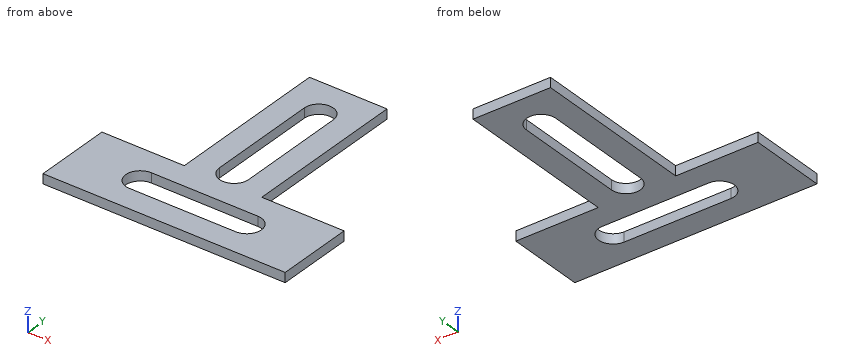
from build123d import *

# Parameters (mm, degrees)
EXTRUDE_2_DEPTH = 2


with BuildPart() as part:
    # 草图1 → 凸台-拉伸2 (new body)
    with BuildSketch(Plane.XY):
        Polygon((25, -8), (-25, -8), (-25, 8), (-8, 8), (-8, 42), (8, 42), (8, 8), (25, 8), align=None)
        with BuildLine():
            Line((-3, 11), (-3, 34))
            ThreePointArc((-3, 34), (0, 37), (3, 34))
            Line((3, 34), (3, 11))
            ThreePointArc((3, 11), (0, 8), (-3, 11))
        make_face(mode=Mode.SUBTRACT)
        with BuildLine():
            Line((-11, 3), (11, 3))
            ThreePointArc((11, 3), (14, 0), (11, -3))
            Line((11, -3), (-11, -3))
            ThreePointArc((-11, -3), (-14, 0), (-11, 3))
        make_face(mode=Mode.SUBTRACT)
    extrude(amount=EXTRUDE_2_DEPTH)


solid = part.part
Can you work these out from the model? Positions are in its coordinate system, mm. Round coordinates to 2 decimals unless told otherwise and drop trailing zeros. Loops run counter-clockwise (first coordinate to the right, second up) from the corner with the lowest first, then second, coordinate; pieces in that order, holes last. Notation, with made-up numbers: (61.5, 81) - (72.5, 81) arc R9 cw to (72.5, 88) - close; hole circle Ø5 at (12.25, 4). An arc over 180 degrees is marked (long way). Write item = value, one per line. Start each with the question number.
(1) If we section it at A-A (y = 30): Please give me the cut outline in (x, z).
(2) If we section it at B-B (z = 0.9): Please give me the cut outline in (x, y), and give its area (3 significant figures).
(3) If we section it at C-C (x = 1.5): Please give me the cut outline in (y, z), and give its area (3 significant figures).
(4) If we section it at D-D (x = 17): Please give me the cut outline in (y, z).
(5) If I drill on probe 1 along X at (y, z) = (34, 1.35); probe 2 along Y at (x, z) = (7, 0.3); probe 3 along Y at (x, z) = (17.5, 1.6), over which ranges is the centre line in solid material (lowest first)? Write a range as [from, to].
(6) For P1, Ø0.6, axis at y = 32, z = 1.5, coming from the +X side; P2, Ø0.6, axis at y = 28, z = 1, coming from the -X side, each with a flat end and sliding along its axis, tell me the tip position at first contact or that it passes through.
Ans:
q1.outline = (-8, 0) - (-3, 0) - (-3, 2) - (-8, 2) - close; (3, 0) - (8, 0) - (8, 2) - (3, 2) - close
q2.outline = (-25, -8) - (25, -8) - (25, 8) - (8, 8) - (8, 42) - (-8, 42) - (-8, 8) - (-25, 8) - close; hole (-11, -3) - (11, -3) arc R3 ccw to (11, 3) - (-11, 3) arc R3 ccw to start; hole (-3, 11) arc R3 ccw to (3, 11) - (3, 34) arc R3 ccw to (-3, 34) - close
q2.area = 1,020 mm²
q3.outline = (-8, 0) - (-3, 0) - (-3, 2) - (-8, 2) - close; (3, 0) - (8.4, 0) - (8.4, 2) - (3, 2) - close; (36.6, 0) - (42, 0) - (42, 2) - (36.6, 2) - close
q3.area = 31.6 mm²
q4.outline = (-8, 0) - (8, 0) - (8, 2) - (-8, 2) - close
q5.probe_1 = [-8, -3], [3, 8]
q5.probe_2 = [-8, -3], [3, 42]
q5.probe_3 = [-8, 8]
q6.P1 = 8
q6.P2 = -8
